For this review, take the finished solid that the model builds, in its own axes (mm). A direction names the side the tool comes from. Round coordinates to 2 decimals unless told otherwise and drop trailing zeros. Write each loop counter-clockwise with the first axis right and the second up, starting at its lowest first coordinate (ties: lowest second). Pieces come first, ordered by that corner, then holes. Notation, with made-up numbers: M -17,-5.75 L -6,-5.75 A19 cw -6,23.25 Z; hole C 41,56 d2. An arc over 180 degrees is marked long. Answer in a Markdown table with one row per item.
```python
from build123d import *

# Parameters (mm, degrees)
SKETCH_1_W           = 200
SKETCH_1_H           = 150
BOSS_EXTRUDE_1_DEPTH = 30
SKETCH_2_R           = 27.5
BOSS_EXTRUDE_2_DEPTH = 30
SKETCH_4_W           = 15
SKETCH_4_H           = 100
BOSS_EXTRUDE_3_DEPTH = 50
SKETCH_5_W           = 200
SKETCH_5_H           = 450
SKETCH_5_R           = 15
BOSS_EXTRUDE_4_DEPTH = 30
FILLET_1_R           = 50


with BuildPart() as part:
    # Sketch 1 → Boss-Extrude 1 (new body)
    with BuildSketch(Plane(origin=(0, 0, 0), x_dir=(1, 0, 0), z_dir=(0, 1, 0))):
        Rectangle(SKETCH_1_W, SKETCH_1_H)
    extrude(amount=BOSS_EXTRUDE_1_DEPTH)

    # Sketch 2 → Boss-Extrude 2 (add)
    with BuildSketch(Plane.XY.offset(75)):
        with BuildLine():
            Line((-58.153846154, 194.769230769), (-100, 30))
            Line((-100, 30), (100, 30))
            Line((100, 30), (58.153846154, 194.769230769))
            ThreePointArc((58.153846154, 194.769230769), (0, 240), (-58.153846154, 194.769230769))
        make_face()
        with Locations((0, 180)):
            Circle(SKETCH_2_R, mode=Mode.SUBTRACT)
    boss_extrude_2 = extrude(amount=-BOSS_EXTRUDE_2_DEPTH)

    # Sketch 4 → Boss-Extrude 3 (add)
    with BuildSketch(Plane.XY.offset(75)):
        with Locations((0, 50)):
            Rectangle(SKETCH_4_W, SKETCH_4_H)
    boss_extrude_3 = extrude(amount=BOSS_EXTRUDE_3_DEPTH)

    # Mirror 1: Boss-Extrude 2, Boss-Extrude 3 across plane
    add(boss_extrude_2.mirror(Plane.XY))
    add(boss_extrude_3.mirror(Plane.XY))

    # Sketch 5 → Boss-Extrude 4 (add)
    with BuildSketch(Plane.XZ):
        Rectangle(SKETCH_5_W, SKETCH_5_H)
        with Locations(Location((0, -175, 0), (0, 0, 270))):
            Circle(SKETCH_5_R, mode=Mode.SUBTRACT)
        with Locations(Location((0, 175, 0), (0, 0, 270))):
            Circle(SKETCH_5_R, mode=Mode.SUBTRACT)
    extrude(amount=-BOSS_EXTRUDE_4_DEPTH)

    # Fillet 1
    fillet_1_edges = [part.edges().sort_by_distance(p)[0] for p in [
        (-100, 15, -225),
        (100, 15, 225),
        (100, 15, -225),
        (-100, 15, 225),
    ]]
    fillet(fillet_1_edges, radius=FILLET_1_R)


solid = part.part
```
Q1. For probe 1 along Z at (x, y) = (54.5, 90.5); probe 2 along Y at (x, z) = (0, -51.5); probe 3 along X at (y, z) = (16, 175), list the stretches that pass through material, from the lowest coordinate up.
Found:
| item | result |
|---|---|
| probe 1 | -75 to -45, 45 to 75 |
| probe 2 | 0 to 152.5, 207.5 to 240 |
| probe 3 | -100 to -15, 15 to 100 |
Q2. Take a section at D-D (y = 180). State the section outline as (x, z) points.
Found:
| item | result |
|---|---|
| outline | M -61.9,-75 L -27.5,-75 L -27.5,-45 L -61.9,-45 Z; M -61.9,45 L -27.5,45 L -27.5,75 L -61.9,75 Z; M 27.5,-75 L 61.9,-75 L 61.9,-45 L 27.5,-45 Z; M 27.5,45 L 61.9,45 L 61.9,75 L 27.5,75 Z |
Q3. Machinability: for faces 4 (the face through (7.5, 65, 100)), 5 (the face through (0, 100, -100)), 6 (the face through (0, 65, 125)), 7 (the face through (-78.784, 113.538, 60.21)), 8 (the face through (-1, 113, 45)), which of the approach directions +Z, -Z, +X, -X, +Y, -Y give a long, thin tool a straight path to every point of the face, cutting with its end or side? Answer none if there is none.
Found:
| item | result |
|---|---|
| face 4 | +Z, +X, +Y |
| face 5 | -Z, +X, -X, +Y |
| face 6 | +Z, +X, -X, +Y |
| face 7 | +Z, -Z, -X, +Y |
| face 8 | +X, -X, +Y |
Q4. Mouldability with a two-part tool opening along Z and no side actions: class faces 1 (the face through (-1, 15, -225)), 2 (the face through (10.138, 14.79, -163.944)), 3 (the face through (12.69, 155.603, -60.21)) as +Z half, -Z half, draft (parallel to the pull), parting line (faces both ways), or undercut.
Found:
| item | result |
|---|---|
| face 1 | -Z half |
| face 2 | undercut |
| face 3 | draft |
Q5. Take a section at C-C (z = -89.5). State the section outline as (x, y) points.
Found:
| item | result |
|---|---|
| outline | M -100,0 L 100,0 L 100,30 L 7.5,30 L 7.5,100 L -7.5,100 L -7.5,30 L -100,30 Z |
Q6. Take a section at A-A (x = 0). State how many separate pieces and enclosed holes the cut face has, then the cut area to 3 significant figures.
Found:
| item | result |
|---|---|
| separate pieces | 5 |
| enclosed holes | 0 |
| area | 28,000 mm² |
Q7. Take a section at B-B (y = 219.5). State the section outline as (x, z) points, then the cut area to 3 significant figures.
Found:
| item | result |
|---|---|
| outline | M -45.16,-75 L 45.16,-75 L 45.16,-45 L -45.16,-45 Z; M -45.16,45 L 45.16,45 L 45.16,75 L -45.16,75 Z |
| area | 5,420 mm² |
Q8. Insertion check: P1, Ø8, axis at x = -33, y = 104.5, coming from the +Z side; P2, Ø1, axis at y = 64.5, z = -60.5, coming from the -X side; P3, Ø25, axis at y = 70.5, z = -106.5, coming from the +X side. Each pin has a flat end and moves straight along its axis. Give the tip position at first contact, or say it passes through.
Found:
| item | result |
|---|---|
| P1 | z = 75 |
| P2 | x = -91.37 |
| P3 | x = 7.5 |
